```python
from build123d import *


with BuildPart() as part:
    # 草图1 → 旋转1 (revolve)
    with BuildSketch(Plane.XY, mode=Mode.PRIVATE) as revolve_1_sk:
        with BuildLine():
            Line((2.5, 0), (4, 0))
            Line((4, 0), (4, 1))
            Line((4, 1), (3, 1))
            Line((3, 1), (3, 2))
            Line((3, 2), (4, 2))
            Line((4, 2), (4, 3))
            Line((4, 3), (3.4, 3))
            Line((3.4, 3), (3.4, 3.1))
            ThreePointArc((3.4, 3.1), (3.136396103, 3.736396103), (2.5, 4))
            Line((2.5, 4), (2.5, 0))
        make_face()
    revolve(revolve_1_sk.sketch.rotate(Axis((0, 0, 0), (0, 1, 0)), 90), axis=Axis((0, 0, 0), (0, 1, 0)))


solid = part.part
```
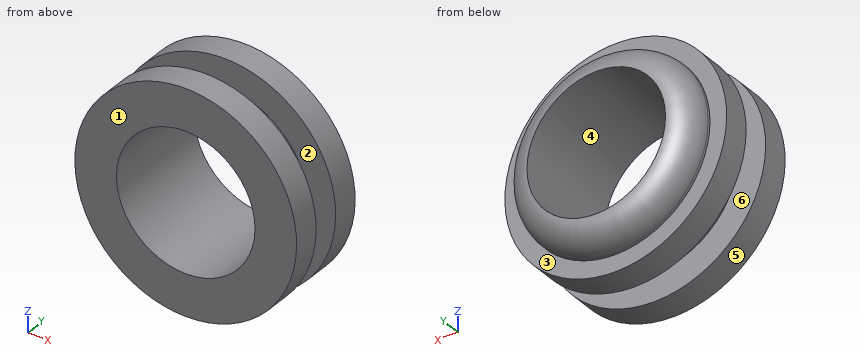
Can you work these out from the model? Positions are in its coordinate system, mm. Face numbers are marked on the shaded views. A direction names the side the tool comes from. Coordinates: 2 decimals unless noted, no trailing zeros. Write each loop counter-clockwise with the first axis right and the second up, starting at its lowest first coordinate (ties: lowest second). Pieces come first, ordered by that corner, then holes. Notation, with made-up numbers: (11, 57) - (68, 57) arc R15 cw to (68, 83) - close; hole circle Ø6 at (-27.5, -5.75). An arc over 180 degrees is marked (long way). Return JSON: item names as keys, results as strings.
Q1. Please list where these lines run through material, in increasing order: L1, parallel to Y at x = 2.75, z = -2.25; L2, parallel to X at y = 3.1, z = 0; L3, parallel to X at y = 2.65, z = 0. Write a range as from..to.
Computed values:
{"L1": "y = 0..1, 2..3", "L2": "x = -3.4..-2.5, 2.5..3.4", "L3": "x = -4..-2.5, 2.5..4"}
Q2. I'm going to push flat-ended pins straight in: pin 1 Ø1 at (x, y) = (-1, 0.5) entering from +Z; pin 2 Ø2 at (x, y) = (-1.5, 3.5) entering from +Z; pin 3 Ø2 at (y, z) = (3, 2.5) entering from -X; pin 4 Ø4 at (x, z) = (1.5, 1.5) entering from -Y. Where does each tip first touch, or does it pass through?
Computed values:
{"pin 1": "stops at z = 3.97", "pin 2": "stops at z = 3.95", "pin 3": "stops at x = -3.71", "pin 4": "stops at y = 0"}
Q3. On a 3-axis mill with a long thin cutter (end or side, diameter ignored), from which of +Z, -Z, +X, -X, +Y, -Y can I reach the whole of each face in a straight line? I mean the marked faces 1, 2 and 3. Say none if no direction works.
Computed values:
{"face 1": "+Z, -Z, +X, -X, -Y", "face 2": "none", "face 3": "+Y"}
Q4. If we section it at B-B (z = 0): Please give me the cut outline in (x, y), then the cut area to 3 significant figures.
Computed values:
{"outline": "(-4, 0) - (-2.5, 0) - (-2.5, 4) arc R0.9 ccw to (-3.4, 3.1) - (-3.4, 3) - (-4, 3) - (-4, 2) - (-3, 2) - (-3, 1) - (-4, 1) - close; (2.5, 0) - (4, 0) - (4, 1) - (3, 1) - (3, 2) - (4, 2) - (4, 3) - (3.4, 3) - (3.4, 3.1) arc R0.9 ccw to (2.5, 4) - close", "area": "8.45 mm2"}
Q5. If we section it at C-C (y = 1.1): Please give me the cut outline in (x, z), then the cut area to 3 significant figures.
Computed values:
{"outline": "circle Ø6 at (0, 0); hole circle Ø5 at (0, 0)", "area": "8.64 mm2"}
Q6. If we section it at D-D (z = 3.5): Please give me the cut outline in (x, y).
Computed values:
{"outline": "(-1.94, 0) - (1.94, 0) - (1.94, 1) - (-1.94, 1) - close; (-1.94, 2) - (1.94, 2) - (1.94, 3) - (-1.94, 3) - close"}
Q7. If we section it at A-A (x = 0): Please give me the cut outline in (y, z).
Computed values:
{"outline": "(0, -4) - (1, -4) - (1, -3) - (2, -3) - (2, -4) - (3, -4) - (3, -3.4) - (3.1, -3.4) arc R0.9 ccw to (4, -2.5) - (0, -2.5) - close; (0, 2.5) - (4, 2.5) arc R0.9 ccw to (3.1, 3.4) - (3, 3.4) - (3, 4) - (2, 4) - (2, 3) - (1, 3) - (1, 4) - (0, 4) - close"}
Q8. Thinking about a two-plate mould opening in Z: for the marked faces 4, 5 and 6, which applies, +Z half, -Z half, draft (parallel to the pull), parting line (faces both ways), or undercut?
Computed values:
{"face 4": "undercut", "face 5": "parting line", "face 6": "draft"}
